```python
from build123d import *

# Parameters (mm, degrees)
SKETCH_1_W             = 80
SKETCH_1_H             = 120
SKETCH_1_W_2           = 76
SKETCH_1_H_2           = 116
EXTRUDE_1_DEPTH        = 315
CUT_EXTRUDE_2_REACH    = 332.492
SKETCH_4_R             = 25
HOLE_WIZARD_M5_1_D     = 5.8
HOLE_WIZARD_M5_1_DEPTH = 2
HOLE_WIZARD_M4_1_D     = 4.8
HOLE_WIZARD_M4_1_DEPTH = 2
CUT_EXTRUDE_3_REACH    = 341.448
SKETCH_15_W            = 50
SKETCH_15_H            = 18
SKETCH_15_W_2          = 60
SKETCH_15_H_2          = 75
FILLET_1_R             = 6


with BuildPart() as part:
    # 草图1 → 拉伸-薄壁1 (new, symmetric)
    with BuildSketch(Plane.XY):
        Rectangle(SKETCH_1_W, SKETCH_1_H)
        Rectangle(SKETCH_1_W_2, SKETCH_1_H_2, mode=Mode.SUBTRACT)
    extrude(amount=EXTRUDE_1_DEPTH, both=True)

    # 草图4 → 切除-拉伸2 (cut, up to next)
    with BuildSketch(Plane.ZY.offset(40), mode=Mode.PRIVATE) as cut_extrude_2_sk1:
        with Locations((0, -20)):
            Circle(SKETCH_4_R)
    cut_extrude_2_tool1 = extrude(cut_extrude_2_sk1.sketch, amount=-CUT_EXTRUDE_2_REACH, mode=Mode.PRIVATE) & part.part
    add(cut_extrude_2_tool1.solids().sort_by_distance((-40, -20, 0))[0], mode=Mode.SUBTRACT)

    # M5 间隙孔1
    with Locations(Plane.ZY.offset(40)):
        with Locations((304.5, 42), (304.5, 28), (304.5, 7.61), (304.5, -6.39), (-304.5, -6.39), (-304.5, 7.61), (-304.5, 28), (-304.5, 42)):
            Hole(HOLE_WIZARD_M5_1_D / 2, depth=HOLE_WIZARD_M5_1_DEPTH)

    # M4 间隙孔1
    with Locations(Plane(origin=(0, 60, 0), x_dir=(1, 0, 0), z_dir=(0, 1, 0))):
        with Locations((-14.175, 246), (10.825, 246), (-14.175, 146), (10.825, 146), (-10.825, -146), (14.175, -146), (-10.825, -246), (14.175, -246)):
            Hole(HOLE_WIZARD_M4_1_D / 2, depth=HOLE_WIZARD_M4_1_DEPTH)

    # 草图15 → 切除-拉伸3 (cut, up to next)
    with BuildSketch(Plane.XZ.offset(60), mode=Mode.PRIVATE) as cut_extrude_3_sk1:
        with Locations((0.475, -273)):
            Rectangle(SKETCH_15_W, SKETCH_15_H)
    cut_extrude_3_tool1 = extrude(cut_extrude_3_sk1.sketch, amount=-CUT_EXTRUDE_3_REACH, mode=Mode.PRIVATE) & part.part
    # 草图15 → 切除-拉伸3 (cut, up to next)
    with BuildSketch(Plane.XZ.offset(60), mode=Mode.PRIVATE) as cut_extrude_3_sk2:
        with Locations((1.975, -171.5)):
            Rectangle(SKETCH_15_W_2, SKETCH_15_H_2)
    cut_extrude_3_tool2 = extrude(cut_extrude_3_sk2.sketch, amount=-CUT_EXTRUDE_3_REACH, mode=Mode.PRIVATE) & part.part
    # 草图15 → 切除-拉伸3 (cut, up to next)
    with BuildSketch(Plane.XZ.offset(60), mode=Mode.PRIVATE) as cut_extrude_3_sk3:
        with Locations((1.975, 171.5)):
            Rectangle(SKETCH_15_W_2, SKETCH_15_H_2)
    cut_extrude_3_tool3 = extrude(cut_extrude_3_sk3.sketch, amount=-CUT_EXTRUDE_3_REACH, mode=Mode.PRIVATE) & part.part
    # 草图15 → 切除-拉伸3 (cut, up to next)
    with BuildSketch(Plane.XZ.offset(60), mode=Mode.PRIVATE) as cut_extrude_3_sk4:
        with Locations((0.475, 273)):
            Rectangle(SKETCH_15_W, SKETCH_15_H)
    cut_extrude_3_tool4 = extrude(cut_extrude_3_sk4.sketch, amount=-CUT_EXTRUDE_3_REACH, mode=Mode.PRIVATE) & part.part
    add(cut_extrude_3_tool1.solids().sort_by_distance((0.475, -60, -273))[0], mode=Mode.SUBTRACT)
    add(cut_extrude_3_tool2.solids().sort_by_distance((1.975, -60, -171.5))[0], mode=Mode.SUBTRACT)
    add(cut_extrude_3_tool3.solids().sort_by_distance((1.975, -60, 171.5))[0], mode=Mode.SUBTRACT)
    add(cut_extrude_3_tool4.solids().sort_by_distance((0.475, -60, 273))[0], mode=Mode.SUBTRACT)

    # 圆角1
    fillet_1_edges = [part.edges().sort_by_distance(p)[0] for p in [
        (25.475, -59, -282),
        (25.475, -59, -264),
        (-24.525, -59, -264),
        (-24.525, -59, -282),
        (-28.025, -59, 134),
        (31.975, -59, 134),
        (31.975, -59, 209),
        (-28.025, -59, 209),
        (-24.525, -59, 282),
        (-24.525, -59, 264),
        (25.475, -59, 264),
        (25.475, -59, 282),
        (31.975, -59, -209),
        (31.975, -59, -134),
        (-28.025, -59, -134),
        (-28.025, -59, -209),
    ]]
    fillet(fillet_1_edges, radius=FILLET_1_R)


solid = part.part
```
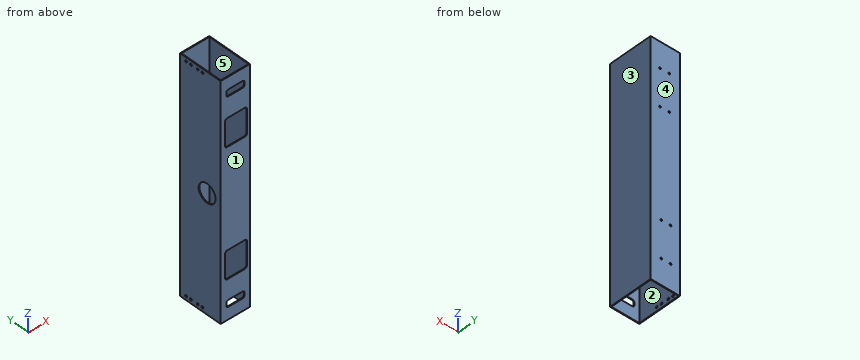
Design review of the part built by this model. Coordinates are the model's own, in mm. Face numbers are marked on the shaded views. A direction names the side the tool comes from. Round coordinates to 2 decimals unless told otherwise and drop trailing zeros. Order: outer loops, then holes, each group sorted by start corner. A loop starts at its lowest first (then second) coordinate and runs counter-clockwise, first axis right, second up. Notation, with made-up numbers: (87, -28) - (116, -28) arc R21 cw to (116, -22) - close; hole circle Ø3 at (78.5, 35). An arc over 180 degrees is marked (long way). Return JSON: item names as keys, results as strings.
Q1. Machinability: for the marked faces 1 and 2, which of the approach directions +Z, -Z, +X, -X, +Y, -Y give a long, thin tool a straight path to every point of the face, cutting with its end or side? Answer none if there is none.
Computed values:
{"face 1": "+Z, -Z, +X, -X, -Y", "face 2": "+Z, -Z"}
Q2. Consider section B-B on z = 226.5. Write out the cut boundary in (x, y).
Computed values:
{"outline": "(-40, -60) - (40, -60) - (40, 60) - (-40, 60) - close; hole (-38, -58) - (38, -58) - (38, 58) - (-38, 58) - close"}
Q3. For pin 1 Ø9.5 at (y, z) = (28, -304.5) entering from -X; pin 2 Ø7.5 at (x, z) = (14.175, 146) entering from -Y; pin 3 Ø5 at (y, z) = (-6.39, -304.5) entering from -X; pin 4 Ø4 at (x, z) = (-14.175, -246) entering from +Y, all flat-tipped, find the tip position at first contact; note any pin that passes through.
Computed values:
{"pin 1": "stops at x = -40", "pin 2": "stops at y = 58", "pin 3": "stops at x = 38", "pin 4": "stops at y = -58"}
Q4. The part is to be moulded in two halves that separate along Y. For the marked faces 3, 4 and 5, say which applies: pulls with the +Y half, pulls with the -Y half, needs draft (parallel to the pull), parting line crosses it, or undercut.
Computed values:
{"face 3": "needs draft", "face 4": "pulls with the +Y half", "face 5": "undercut"}
Q5. Consider section A-A on y = -20. Write out the cut boundary in (x, z), plus the area to 3 significant figures.
Computed values:
{"outline": "(-40, -315) - (-38, -315) - (-38, -25) - (-40, -25) - close; (-40, 25) - (-38, 25) - (-38, 315) - (-40, 315) - close; (38, -315) - (40, -315) - (40, 315) - (38, 315) - close", "area": "2,420 mm2"}
Q6. Wall thickness on L1, parallel to X at y = 58.95, z = -146 (3 decimals); L2, parallel to Y at x = 7, z = -104; L3, parallel to X at y = -8, z = 53.5: over which ranges is each line inside the solid? List them lowest first. Write a range as [from, to].
Computed values:
{"L1": "x = [-40, -16.575], [-11.775, 8.425], [13.225, 40]", "L2": "y = [-60, -58], [58, 60]", "L3": "x = [-40, -38], [38, 40]"}
